Source: three-view drawing plus pictorial views. Frame: mm from the lowest corner of the part. A direction names the side the tool comes from. Give positions to 0.01 mm unless a question says otherwise; leave off trailing zeros. Order: outer loops, then holes, each group sorted by start corner. A loop starts at its lowest first (then second) coordinate and runs counter-clockwise, first axis right, second up.
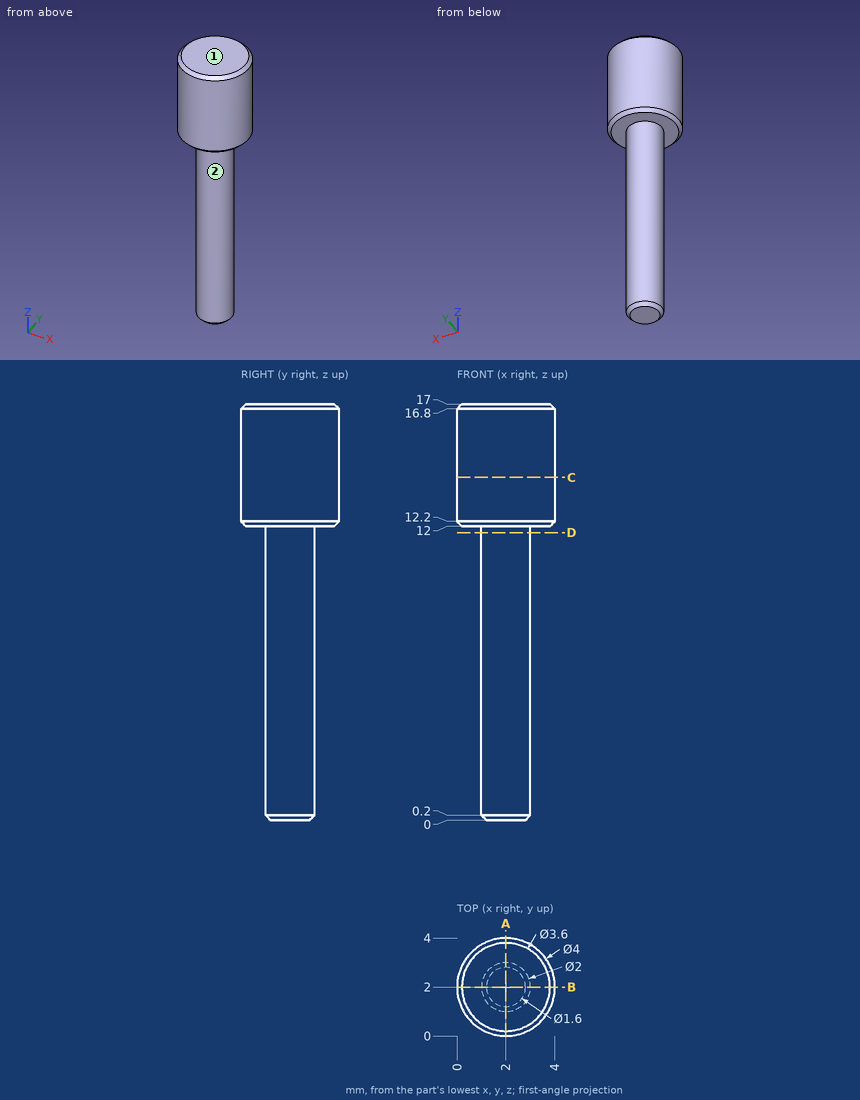
(1) Section D-D, the plane z = 11.75. Return loops of the section in (x, y), plus the area to 3 significant figures.
(2) Access query for the marked faces 1 and 2. Directions: +Z, -Z, +X, -X, +Y, -Y. A direction counts if a zero-diameter tool reaches every point of the face in a straight line with its end or side. Return the directions, or none.
(3) Section C-C, the plane z = 14. Return loops of the section in (x, y).
(4) Section A-A, the plane x = 2. Return loops of the section in (y, z), plus the area to 3 significant figures.
(5) Line query: line 1 along Z through (x, y) = (3.15, 1.1); line 2 along Y through (x, z) = (1.4, 7); line 3 along X through (y, z) = (2.1, 15.25). Output: solid intervals per line, ascending.
(6) Pin query (flat end, axial travel): pin 1 Ø1 at (x, z) = (0.5, 12.5) entering from +Y; pin 2 Ø1 at (y, z) = (2, 2.5) entering from -X. Return the tip coordinate at first contact, or that it passes through.
Checks:
1. outline: circle Ø2 at (2, 2)
1. area: 3.14 mm2
2. face 1: +Z, +X, -X, +Y, -Y
2. face 2: -Z
3. outline: circle Ø4 at (2, 2)
4. outline: (0, 12.2) - (0.2, 12) - (1, 12) - (1, 0.2) - (1.2, 0) - (2.8, 0) - (3, 0.2) - (3, 12) - (3.8, 12) - (4, 12.2) - (4, 16.8) - (3.8, 17) - (0.2, 17) - (0, 16.8) - close
4. area: 43.9 mm2
5. line 1: z = 12 to 17
5. line 2: y = 1.2 to 2.8
5. line 3: x = 0 to 4
6. pin 1: stops at y = 3.73
6. pin 2: stops at x = 1
